Part model, mm, in its own coordinate system. A direction names the side the tool comes from. Round coordinates to 2 decimals unless told otherwise and drop trailing zeros. Loops run counter-clockwise (first coordinate to the right, second up) from the corner with the lowest first, then second, coordinate; pieces in that order, holes last. Notation, with made-up numbers: M 88.5,-34 L 92.5,-34 A16 ccw 92.5,-16 Z; hole C -36,5.5 d10. An arc over 180 degrees is marked long. Put each result on its own line as item: value. Start each with the question number.
1) Slice it at C-C on y = 2.75. Give the cut face in (x, z), then the cut area to 3 significant figures.
2) Probe line 1 along X through (y, z) = (20.25, 110); line 2 along Z through (x, y) = (15.9, 10.5); line 3 along Y through (x, z) = (-7.5, 44). List the from-to ranges inside material, lowest first.
3) Slice it at B-B on z = 43.5. Give the cut face in (x, y), then the cut area to 3 significant figures.
4) Slice it at D-D on z = 116. Give the cut face in (x, y), then the cut area to 3 significant figures.
5) Which spindle directions (+Z, -Z, +X, -X, +Y, -Y) get a long thin tool onto all of the face, cutting with end or side? Do faces 1 (the flat face through (0, -1, 25)), 2 (the flat face through (16, 11, 0)). Say none if no direction does.
6) Slice it at A-A on y = 10.5. Give the cut face in (x, z).
7) Pull direction Y, two halves, no side cores. Call faces 3 (the flat face through (0, 0, 72)), 4 (the cylindrical face through (-16, 8.9, 23.8)), 5 (the flat face through (15, 10, 59)): +Y half, -Y half, draft (parallel to the pull), parting line (faces both ways), or undercut.
8) Drop flat-ended pins along their axis: pin 1 Ø5 at (x, z) = (-9.93, 116) entering from +Y; pin 2 Ø2 at (x, y) = (2, -1) entering from -Z; pin 3 Ø2 at (x, y) = (-13.5, 19) entering from +Z. Give the stop position or say it passes through.
```python
from build123d import *

# Parameters (mm, degrees)
BOSS_EXTRUDE1_DEPTH = 120
SKETCH2_R           = 2
CUT_EXTRUDE1_DEPTH  = 124.749747474
SKETCH3_W           = 30
SKETCH3_H           = 25
CUT_EXTRUDE2_DEPTH  = 124.3612581
SKETCH4_R           = 2
CUT_EXTRUDE3_DEPTH  = 127.82665335


with BuildPart() as part:
    # Sketch1 → Boss-Extrude1 (new body)
    with BuildSketch(Plane.XY):
        Polygon((-15, 23), (-15, 0), (15, 0), (15, 23), (17, 23), (17, -2), (-17, -2), (-17, 23), align=None)
    extrude(amount=BOSS_EXTRUDE1_DEPTH)

    # Sketch2 → Cut-Extrude1 (cut, through all)
    with BuildSketch(Plane.XZ.offset(2)):
        with Locations((0.071255778, 98.679491924)):
            Circle(SKETCH2_R)
        with Locations((10.071255778, 116)):
            Circle(SKETCH2_R)
        with Locations((-9.928744222, 116)):
            Circle(SKETCH2_R)
    extrude(amount=-CUT_EXTRUDE1_DEPTH, mode=Mode.SUBTRACT)

    # Sketch3 → Cut-Extrude2 (cut, through all)
    with BuildSketch(Plane(origin=(0, 0, 0), x_dir=(1, 0, 0), z_dir=(0, 1, 0))):
        with Locations((0, -12.5)):
            Rectangle(SKETCH3_W, SKETCH3_H)
    extrude(amount=-CUT_EXTRUDE2_DEPTH, mode=Mode.SUBTRACT)

    # Sketch4 → Cut-Extrude3 (cut, through all)
    with BuildSketch(Plane(origin=(17, 0, 0), x_dir=(0, 0, -1), z_dir=(1, 0, 0))):
        with Locations(Location((-25, 10.5, 0), (0, 0, 90))):
            Circle(SKETCH4_R)
    extrude(amount=-CUT_EXTRUDE3_DEPTH, mode=Mode.SUBTRACT)


solid = part.part
```
Recorded:
1. outline: M -17,0 L -15,0 L -15,120 L -17,120 Z; M 15,0 L 17,0 L 17,120 L 15,120 Z
1. area: 480 mm2
2. line 1: x = -17 to -15, 15 to 17
2. line 2: z = 0 to 23, 27 to 120
2. line 3: y = -2 to 0
3. outline: M -17,-2 L 17,-2 L 17,23 L 15,23 L 15,0 L -15,0 L -15,23 L -17,23 Z
3. area: 160 mm2
4. outline: M -17,-2 L -11.93,-2 L -11.93,0 L -15,0 L -15,23 L -17,23 Z; M -7.93,-2 L 8.07,-2 L 8.07,0 L -7.93,0 Z; M 12.07,-2 L 17,-2 L 17,23 L 15,23 L 15,0 L 12.07,0 Z
4. area: 144 mm2
5. face 1: -Z, +Y, -Y
5. face 2: -Z, +X, -X, +Y, -Y
6. outline: M -17,0 L -15,0 L -15,23 L -17,23 Z; M -17,27 L -15,27 L -15,120 L -17,120 Z; M 15,0 L 17,0 L 17,23 L 15,23 Z; M 15,27 L 17,27 L 17,120 L 15,120 Z
7. face 3: +Y half
7. face 4: undercut
7. face 5: draft
8. pin 1: stops at y = 0
8. pin 2: stops at z = 25
8. pin 3: passes through
